Work out the finished part from the listing and answer in its coordinate system (mm). A direction names the side the tool comes from. Coordinates: 2 decimals unless noted, no trailing zeros. Write each loop counter-clockwise with the first axis right and the second up, starting at its lowest first coordinate (ties: lowest second). Pieces come first, ordered by that corner, then holes. Notation, with made-up numbers: (-7.75, 66.5) - (-0.75, 66.5) arc R11 cw to (-0.75, 75.5) - close; hole circle Ø3 at (-39, -4.75). An arc over 180 degrees is marked (long way). Answer as a JSON object with one key per item and string values. Group by question number.
from build123d import *

# Parameters (mm, degrees)
BASE_BLOCK_DEPTH                 = 20
CENTER_POCKET_SKETCH_OUTSIDE_W   = 112.322
CENTER_POCKET_SKETCH_OUTSIDE_H   = 62.322
CENTER_POCKET_CUT_DEPTH          = 40
MOUNTING_HOLES_SKETCH_R          = 2.25
MOUNTING_HOLES_4_5_DEPTH         = 40
SADDLE_CUT_A_DEPTH               = 55
SADDLE_CUT_B_DEPTH               = 110
SADDLE_MIRROR_RIGHT_COPY_1_DEPTH = 110


with BuildPart() as part:
    # Base Profile Sketch → Base Block (new, symmetric)
    with BuildSketch(Plane.XY):
        Polygon((-35, 18.587360595), (-25, 18.587360595), (-10, 18.587360595), (10, 18.587360595), (25, 18.587360595), (35, 18.587360595), (35, 8.587360595), (45, 8.587360595), (45, -6.412639405), (22.5, -6.412639405), (27.5, -1.412639405), (-27.5, -1.412639405), (-22.5, -6.412639405), (-45, -6.412639405), (-45, 8.587360595), (-35, 8.587360595), align=None)
    extrude(amount=BASE_BLOCK_DEPTH, both=True)

    # Center Pocket Sketch outside → Center Pocket Cut (cut)
    with BuildSketch(Plane(origin=(0, 18.587360595, 0), x_dir=(1, 0, 0), z_dir=(0, 1, 0))):
        Rectangle(CENTER_POCKET_SKETCH_OUTSIDE_W, CENTER_POCKET_SKETCH_OUTSIDE_H)
        Polygon((30, 20), (-30, 20), (-30, 15), (-45, 15), (-45, -15), (-30, -15), (-30, -20), (30, -20), (30, -15), (45, -15), (45, 15), (30, 15), align=None, mode=Mode.SUBTRACT)
    extrude(amount=-CENTER_POCKET_CUT_DEPTH, mode=Mode.SUBTRACT)

    # Mounting Holes Sketch → Mounting Holes _4.5 (cut)
    with BuildSketch(Plane(origin=(0, 18.587360595, 0), x_dir=(1, 0, 0), z_dir=(0, 1, 0))):
        with Locations(Location((-30, 7.5, 0), (0, 0, 270))):
            Circle(MOUNTING_HOLES_SKETCH_R)
        with Locations(Location((-30, -7.5, 0), (0, 0, 180))):
            Circle(MOUNTING_HOLES_SKETCH_R)
        with Locations(Location((30, -7.5, 0), (0, 0, 270))):
            Circle(MOUNTING_HOLES_SKETCH_R)
        with Locations(Location((30, 7.5, 0), (0, 0, 180))):
            Circle(MOUNTING_HOLES_SKETCH_R)
        with Locations(Location((0, 15, 0), (0, 0, 270))):
            Circle(MOUNTING_HOLES_SKETCH_R)
        with Locations(Location((0, -15, 0), (0, 0, 180))):
            Circle(MOUNTING_HOLES_SKETCH_R)
    extrude(amount=-MOUNTING_HOLES_4_5_DEPTH, mode=Mode.SUBTRACT)

    # Saddle Profile Sketch → Saddle Cut A (cut, symmetric)
    with BuildSketch(Plane.XY.offset(15)):
        with BuildLine():
            Line((-10, 18.587360595), (-25, 18.587360595))
            ThreePointArc((-25, 18.587360595), (-17.5, 11.087360595), (-10, 18.587360595))
        make_face()
    saddle_cut_a = extrude(amount=SADDLE_CUT_A_DEPTH, both=True, mode=Mode.SUBTRACT)

    # Sketch5_7 → Saddle Cut B (cut)
    with BuildSketch(Plane.XY.offset(15)):
        with BuildLine():
            ThreePointArc((-17.5, 6.087360595), (-26.338834765, 9.74852583), (-30, 18.587360595))
            Line((-30, 18.587360595), (-30, -6.412639405))
            Line((-30, -6.412639405), (-22.5, -6.412639405))
            Line((-22.5, -6.412639405), (-27.5, -1.412639405))
            Line((-27.5, -1.412639405), (-7.5, -1.412639405))
            Line((-7.5, -1.412639405), (-7.5, 6.087360595))
            Line((-7.5, 6.087360595), (-17.5, 6.087360595))
        make_face()
    saddle_cut_b = extrude(amount=SADDLE_CUT_B_DEPTH, mode=Mode.SUBTRACT)

    # Saddle Mirror Front: Saddle Cut B across plane
    add(saddle_cut_b.mirror(Plane.XY), mode=Mode.SUBTRACT)

    # Saddle Mirror Right: Saddle Cut A, Saddle Cut B across plane
    add(saddle_cut_a.mirror(Plane(origin=(0, 0, 0), x_dir=(0, 0, 1), z_dir=(1, 0, 0))), mode=Mode.SUBTRACT)
    add(saddle_cut_b.mirror(Plane(origin=(0, 0, 0), x_dir=(0, 0, 1), z_dir=(1, 0, 0))), mode=Mode.SUBTRACT)

    # Saddle Mirror Right copy 1 sketch → Saddle Mirror Right copy 1 (cut)
    with BuildSketch(Plane(origin=(0, 0, -15), x_dir=(-1, 0, 0), z_dir=(0, 0, -1))):
        with BuildLine():
            ThreePointArc((-17.5, 6.087360595), (-26.338834765, 9.74852583), (-30, 18.587360595))
            Line((-30, 18.587360595), (-30, -6.412639405))
            Line((-30, -6.412639405), (-22.5, -6.412639405))
            Line((-22.5, -6.412639405), (-27.5, -1.412639405))
            Line((-27.5, -1.412639405), (-7.5, -1.412639405))
            Line((-7.5, -1.412639405), (-7.5, 6.087360595))
            Line((-7.5, 6.087360595), (-17.5, 6.087360595))
        make_face()
    extrude(amount=SADDLE_MIRROR_RIGHT_COPY_1_DEPTH, mode=Mode.SUBTRACT)


solid = part.part
Q1. Section A-A on x = 0 is taken. Determine the outline of the cut face in (y, z).
Q2. Section B-B on y = -3.25 is taken. Determine the outline of the cut face in (x, z).
Q3. Section D-D on y = 5.25 is taken. Determine the outline of the cut face in (x, z), plus the area to 3 significant figures.
Q4. Section C-C on z = -7.5 is taken. Determine the outline of the cut face in (x, y), plus the area to 3 significant figures.
Q5. Consider L1, parallel to Z at x = 29, y = -4; L2, parallel to Z at x = -1, y = 15.5; L3, parallel to Z at x = 10, y = 3.5. Determine where each line is inside the solid, lowest interval first. Write a range as from..to.
Q6. For a pull along Z with two mould halves and no side action, classify faces 1 (the face through (0, 9, 20)), 2 (the face through (-31.369, 6.262, -9.286)), 3 (the face through (34, -6.413, 0)) as +Z half, -Z half, draft (parallel to the pull), parting line (faces both ways), or undercut.
Q7. Flat-ended cylindrical pins translate along their axes: pin 1 Ø5.5 at (x, z) = (-14, 17.5) entering from -Y; pin 2 Ø2.5 at (x, z) = (12.5, 17.5) entering from -Y; pin 3 Ø2.5 at (y, z) = (1.5, -16.5) entering from +X. Find the tip coordinate at first contact, or state that the pin passes through.
Q8. A tool of negligible diameter and unlimited length cuts with its end or side. For faces 4 (the face through (12, 6.087, -17)), 5 (the face through (-26.24, 9.65, -17.46)), 6 (the face through (-40, 8.587, 0)), from which of +Z, -Z, +X, -X, +Y, -Y can it reach the whole face along a straight path? Write none if from no direction.
Numbers:
{
 "1": {"outline": "(-1.41, -20) - (18.59, -20) - (18.59, -17.25) - (-1.41, -17.25) - close; (-1.41, -12.75) - (18.59, -12.75) - (18.59, 12.75) - (-1.41, 12.75) - close; (-1.41, 17.25) - (18.59, 17.25) - (18.59, 20) - (-1.41, 20) - close"},
 "2": {"outline": "(-45, -15) - (-25.66, -15) - (-25.66, 15) - (-45, 15) - close; (25.66, -15) - (45, -15) - (45, 15) - (25.66, 15) - close; hole circle Ø4.5 at (-30, -7.5); hole circle Ø4.5 at (-30, 7.5); hole circle Ø4.5 at (30, -7.5); hole circle Ø4.5 at (30, 7.5)"},
 "3": {"outline": "(-45, -15) - (-7.5, -15) - (-7.5, -20) - (7.5, -20) - (7.5, -15) - (45, -15) - (45, 15) - (7.5, 15) - (7.5, 20) - (-7.5, 20) - (-7.5, 15) - (-45, 15) - close; hole circle Ø4.5 at (-30, -7.5); hole circle Ø4.5 at (-30, 7.5); hole circle Ø4.5 at (0, -15); hole circle Ø4.5 at (0, 15); hole circle Ø4.5 at (30, -7.5); hole circle Ø4.5 at (30, 7.5)", "area": "2,750 mm²"},
 "4": {"outline": "(-45, -6.41) - (-32.25, -6.41) - (-32.25, 18.59) - (-35, 18.59) - (-35, 8.59) - (-45, 8.59) - close; (-27.75, -6.41) - (-22.5, -6.41) - (-27.5, -1.41) - (27.5, -1.41) - (22.5, -6.41) - (27.75, -6.41) - (27.75, 18.59) - (25, 18.59) arc R7.5 cw to (10, 18.59) - (-10, 18.59) arc R7.5 cw to (-25, 18.59) - (-27.75, 18.59) - close; (32.25, -6.41) - (45, -6.41) - (45, 8.59) - (35, 8.59) - (35, 18.59) - (32.25, 18.59) - close", "area": "1,400 mm²"},
 "5": {"L1": "z = -15..-9.52, -5.48..5.48, 9.52..15", "L2": "z = -20..-17.02, -12.98..12.98, 17.02..20", "L3": "z = -15..15"},
 "6": {"face 1": "+Z half", "face 2": "undercut", "face 3": "draft"},
 "7": {"pin 1": "stops at y = -1.41", "pin 2": "stops at y = 6.09", "pin 3": "stops at x = 7.5"},
 "8": {"face 4": "-Z, +X, -Y", "face 5": "-Z, -X, -Y", "face 6": "+Z, -Z, -X, +Y"}
}
